Geometry check sheet. Reference: drawing and pictorial views, mm from the part's lowest x, y, z. Round coordinates to 2 decimals unless told otherwise and drop trailing zeros. Order: outer loops, then holes, each group sorted by start corner. A loop starts at its lowest first (then second) coordinate and runs counter-clockwise, first axis right, second up.
(1) Draft check along X on the marked faces 1 and 2. Enter one of: pulls with the +X half, pulls with the -X half, needs draft (parallel to the pull), parting line crosses it, or undercut.
(2) Cross-section at A-A on z = 25. Enter the section's corners in (x, y).
(3) Cross-section at B-B on y = 20. Enter the section's corners in (x, z), and give its area (3 significant figures).
(4) Thickness scan on L1, parallel to Y at x = 0.9, z = 25. Record the ranges inside material, lowest first.
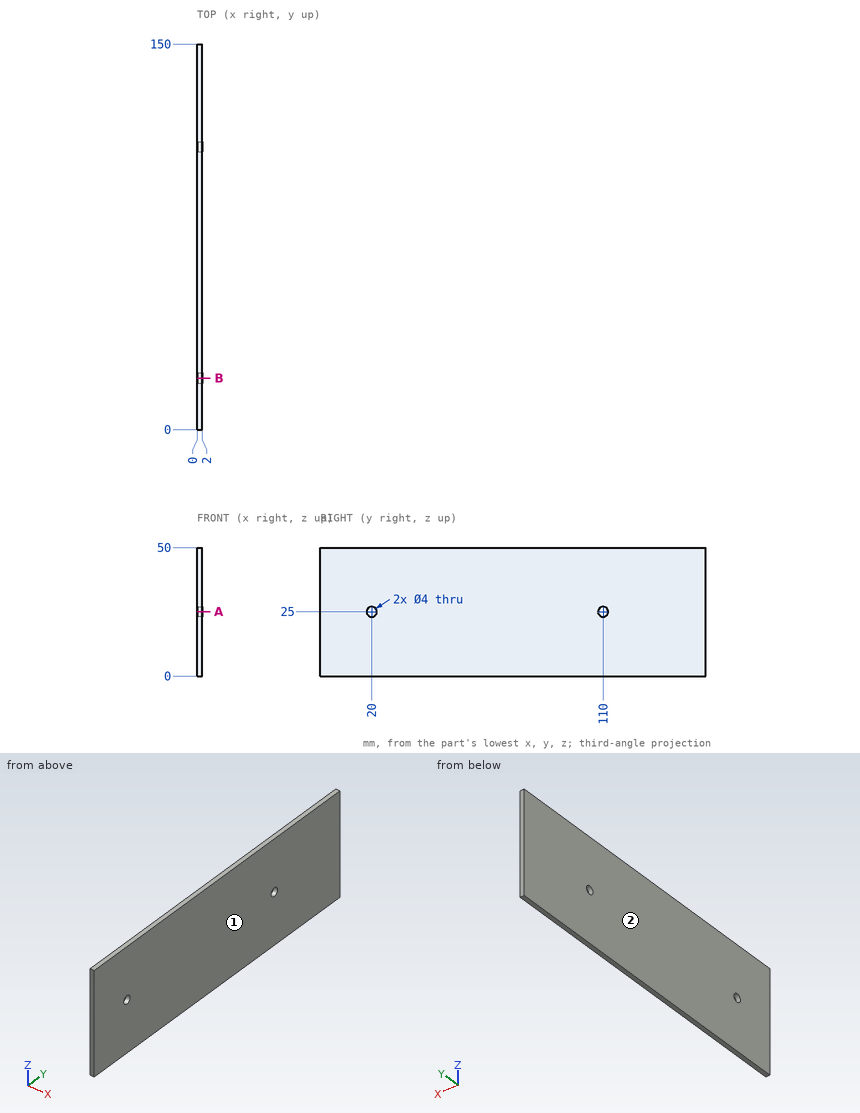
Found:
1. face 1: pulls with the +X half
1. face 2: pulls with the -X half
2. outline: (0, 0) - (2, 0) - (2, 18) - (0, 18) - close; (0, 22) - (2, 22) - (2, 108) - (0, 108) - close; (0, 112) - (2, 112) - (2, 150) - (0, 150) - close
3. outline: (0, 0) - (2, 0) - (2, 23) - (0, 23) - close; (0, 27) - (2, 27) - (2, 50) - (0, 50) - close
3. area: 92.0 mm2
4. L1: y = 0 to 18, 22 to 108, 112 to 150
